from build123d import *


with BuildPart() as part:
    # Sketch2 → Revolve1 (revolve)
    with BuildSketch(Plane.XY, mode=Mode.PRIVATE) as revolve1_sk:
        Polygon((0, 137), (0, 202), (30, 202), (30, 190), (16, 190), (16, 176), (30, 176), (30, 164), (16, 164), (16, 150), (63, 150), (63, 104), (49, 104), (49, 137), align=None)
    revolve(revolve1_sk.sketch.rotate(Axis((0, 0, 0), (1, 0, 0)), 90), axis=Axis((0, 0, 0), (1, 0, 0)))


solid = part.part
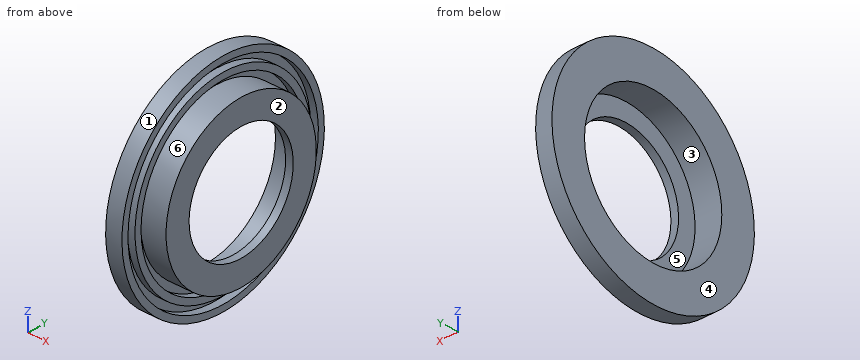
Source: CAD feature listing. Evaluate the final solid. Frame: model axes, mm. Face numbers are marked on the shaded views. A direction names the side the tool comes from. Round coordinates to 2 decimals unless told otherwise and drop trailing zeros. Loops run counter-clockwise (first coordinate to the right, second up) from the corner with the lowest first, then second, coordinate; pieces in that order, holes last. Notation, with made-up numbers: (20.25, 2) -> (73.25, 2) arc R8 ccw to (73.25, 11) -> close; hole circle Ø9 at (-12.75, 33.5). An arc over 180 degrees is marked (long way). Answer as a JSON object with one key per item and string values. Group by question number.
Q1. Section query A-A (y = 0). Output: boundary loops of the cut face in (x, z).
Q2. Section query D-D (x = 9.5). Output: boundary loops of the cut face in (y, z).
Q3. Mould query, pull axis Z, two halves, no side actions, for the marked faces 1, 2 and 3. Classes: pulls with the +Z half, pulls with the -Z half, needs draft (parallel to the pull), parting line crosses it, or undercut.
Q4. Contact query for flat-ended pins moving along their axis: P1, Ø1.5, axis at x = 23.5, y = -109.5, coming from the +Z side; P2, Ø3, axis at x = 55.5, y = -5, coming from the +Z side; P3, Ø8, axis at y = -75.5, z = -141.5, coming from the +X side. Output: stop coordinate, or through.
Q5. Section query C-C (x = 42). Output: boundary loops of the cut face in (y, z).
Q6. Ray query, line 1 (Y direction, x = 25.25, z = 0); line 2 (Y direction, x = 23.5, z = -56); line 3 (Y direction, x = 52.25, z = 0). Return the intervals inside material, ascending. Write a range as from..to.
Q7. Access query for the marked faces 4, 5 and 6. Directions: +Z, -Z, +X, -X, +Y, -Y. A direction counts if a zero-diameter tool reaches every point of the face in a straight line with its end or side. Return the directions, or none.
Completed:
{
 "1": {"outline": "(0, -202) -> (30, -202) -> (30, -190) -> (16, -190) -> (16, -176) -> (30, -176) -> (30, -164) -> (16, -164) -> (16, -150) -> (63, -150) -> (63, -104) -> (49, -104) -> (49, -137) -> (0, -137) -> close; (0, 137) -> (49, 137) -> (49, 104) -> (63, 104) -> (63, 150) -> (16, 150) -> (16, 164) -> (30, 164) -> (30, 176) -> (16, 176) -> (16, 190) -> (30, 190) -> (30, 202) -> (0, 202) -> close"},
 "2": {"outline": "circle Ø404 at (0, 0); hole circle Ø274 at (0, 0)"},
 "3": {"face 1": "parting line crosses it", "face 2": "needs draft", "face 3": "undercut"},
 "4": {"P1": "z = 170.23", "P2": "z = 149.96", "P3": "x = 30"},
 "5": {"outline": "circle Ø300 at (0, 0); hole circle Ø274 at (0, 0)"},
 "6": {"line 1": "-202..-190, -176..-164, -150..-137, 137..150, 164..176, 190..202", "line 2": "-194.08..-181.56, -166.85..-154.14, -139.15..-125.03, 125.03..139.15, 154.14..166.85, 181.56..194.08", "line 3": "-150..-104, 104..150"},
 "7": {"face 4": "+Z, -Z, -X, +Y, -Y", "face 5": "-X", "face 6": "+X"}
}
